Source: three-view drawing plus pictorial views. Frame: mm from the lowest corner of the part. Round coordinates to 2 decimals unless told otherwise and drop trailing zeros. Loops run counter-clockwise (first coordinate to the right, second up) from the corner with the lowest first, then second, coordinate; pieces in that order, holes last. Notation, with made-up numbers: M 62.5,-38.5 L 82.5,-38.5 A33 cw 82.5,-6.5 Z; hole C 58,38 d11. An arc over 180 degrees is marked long. Write each question's results on one line, items separated by ' | '.
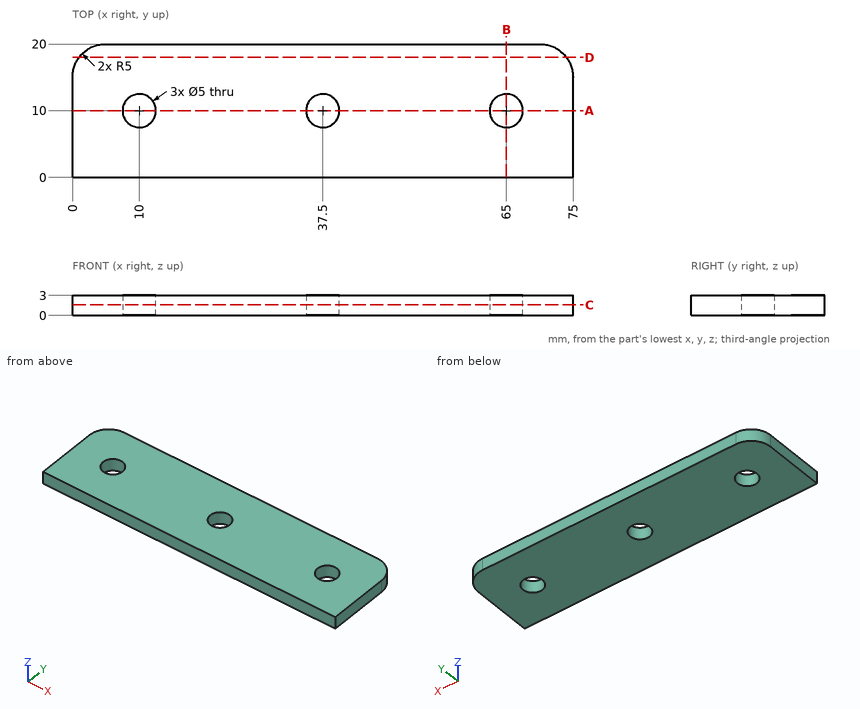
1. Ray query, probe 1 along Y at (x, z) = (10, 2.35); probe 2 along X at (y, z) = (11, 2.55); probe 3 along Y at (x, z) = (64.5, 2.9). Return the intervals inside material, ascending.
Answer key:
probe 1: y = 0 to 7.5, 12.5 to 20 | probe 2: x = 0 to 7.71, 12.29 to 35.21, 39.79 to 62.71, 67.29 to 75 | probe 3: y = 0 to 7.55, 12.45 to 20
2. Section C-C (z = 1.6). Output: boundary loops of the cut face in (x, y).
Answer key:
outline: M 0,0 L 75,0 L 75,15 A5 ccw 70,20 L 5,20 A5 ccw 0,15 Z; hole C 10,10 d5; hole C 37.5,10 d5; hole C 65,10 d5
3. Pin query (flat end, axial travel): P1, Ø4.5, axis at x = 65, y = 10, coming from the -Z side; P2, Ø1, axis at x = 43, y = 10.5, coming from the -Z side. Return the tip coordinate at first contact, or that it passes through.
Answer key:
P1: passes through | P2: stops at z = 0
4. Section D-D (y = 18). Output: boundary loops of the cut face in (x, z).
Answer key:
outline: M 1,0 L 74,0 L 74,3 L 1,3 Z
5. Section A-A (y = 10). Output: boundary loops of the cut face in (x, z).
Answer key:
outline: M 0,0 L 7.5,0 L 7.5,3 L 0,3 Z; M 12.5,0 L 35,0 L 35,3 L 12.5,3 Z; M 40,0 L 62.5,0 L 62.5,3 L 40,3 Z; M 67.5,0 L 75,0 L 75,3 L 67.5,3 Z
6. Section B-B (x = 65). Output: boundary loops of the cut face in (y, z).
Answer key:
outline: M 0,0 L 7.5,0 L 7.5,3 L 0,3 Z; M 12.5,0 L 20,0 L 20,3 L 12.5,3 Z
